Model file for the job. Use its own axes, mm. A direction names the side the tool comes from. Coordinates: 2 decimals unless noted, no trailing zeros. Order: outer loops, then holes, each group sorted by start corner. A loop starts at its lowest first (then second) coordinate and runs counter-clockwise, first axis right, second up.
from build123d import *

# Parameters (mm, degrees)
BASE_PLATE_SKETCH_W = 88
BASE_PLATE_SKETCH_H = 110
BASE_PLATE_DEPTH    = 18
SIDE_BOSS_SKETCH_W  = 88
SIDE_BOSS_SKETCH_H  = 6
SIDE_BOSS_DEPTH     = 75
REAR_BOSS_SKETCH_R  = 9.5
REAR_BOSS_DEPTH     = 12
ANGLED_CUT_REACH    = 137.133
ANGLED_CUT_SKETCH_R = 5
ARCH_CUT_SKETCH_R   = 24
ARCH_CUT_DEPTH      = 93.743251702


with BuildPart() as part:
    # Base Plate Sketch → Base Plate (new body)
    with BuildSketch(Plane.XY):
        with Locations((0, 55)):
            Rectangle(BASE_PLATE_SKETCH_W, BASE_PLATE_SKETCH_H)
    extrude(amount=-BASE_PLATE_DEPTH)

    # Side Boss Sketch → Side Boss (add)
    with BuildSketch(Plane(origin=(0, 0, 0), x_dir=(1, 0, 0), z_dir=(0, 1, 0))):
        with Locations((0, 21)):
            Rectangle(SIDE_BOSS_SKETCH_W, SIDE_BOSS_SKETCH_H)
    extrude(amount=SIDE_BOSS_DEPTH)

    # Rear Boss Sketch → Rear Boss (add)
    with BuildSketch(Plane.XZ):
        with BuildLine():
            Line((-44, -24), (-19.769224603, -55.302867659))
            ThreePointArc((-19.769224603, -55.302867659), (0, -65), (19.769224603, -55.302867659))
            Line((19.769224603, -55.302867659), (44, -24))
            Line((44, -24), (-44, -24))
        make_face()
        with Locations(Location((0, -40, 0), (0, 0, 270))):
            Circle(REAR_BOSS_SKETCH_R, mode=Mode.SUBTRACT)
    extrude(amount=-REAR_BOSS_DEPTH)

    # Angled Cut: up to this face of the body (flat: up to its plane)
    angled_cut_end = Plane(part.part.faces().sort_by_distance((0, 43.5, -24))[0])
    # Angled Cut Sketch → Angled Cut (cut, up to the picked face)
    with BuildSketch(Plane.XY, mode=Mode.PRIVATE) as angled_cut_sk1:
        with Locations((-27.5, 95)):
            Circle(ANGLED_CUT_SKETCH_R)
    angled_cut_tool1 = split(extrude(angled_cut_sk1.sketch, amount=-ANGLED_CUT_REACH, mode=Mode.PRIVATE), bisect_by=angled_cut_end, keep=Keep.BOTH, mode=Mode.PRIVATE)
    # Angled Cut Sketch → Angled Cut (cut, up to the picked face)
    with BuildSketch(Plane.XY, mode=Mode.PRIVATE) as angled_cut_sk2:
        with Locations((27.5, 95)):
            Circle(ANGLED_CUT_SKETCH_R)
    angled_cut_tool2 = split(extrude(angled_cut_sk2.sketch, amount=-ANGLED_CUT_REACH, mode=Mode.PRIVATE), bisect_by=angled_cut_end, keep=Keep.BOTH, mode=Mode.PRIVATE)
    # Angled Cut Sketch → Angled Cut (cut, up to the picked face)
    with BuildSketch(Plane.XY, mode=Mode.PRIVATE) as angled_cut_sk3:
        with Locations((29.652920455, 60)):
            Circle(ANGLED_CUT_SKETCH_R)
    angled_cut_tool3 = split(extrude(angled_cut_sk3.sketch, amount=-ANGLED_CUT_REACH, mode=Mode.PRIVATE), bisect_by=angled_cut_end, keep=Keep.BOTH, mode=Mode.PRIVATE)
    # Angled Cut Sketch → Angled Cut (cut, up to the picked face)
    with BuildSketch(Plane.XY, mode=Mode.PRIVATE) as angled_cut_sk4:
        with Locations((-29.652920455, 60)):
            Circle(ANGLED_CUT_SKETCH_R)
    angled_cut_tool4 = split(extrude(angled_cut_sk4.sketch, amount=-ANGLED_CUT_REACH, mode=Mode.PRIVATE), bisect_by=angled_cut_end, keep=Keep.BOTH, mode=Mode.PRIVATE)
    add(angled_cut_tool1.solids().sort_by(Axis((-27.5, 95, 0), (0, 0, -1)))[0], mode=Mode.SUBTRACT)
    add(angled_cut_tool2.solids().sort_by(Axis((27.5, 95, 0), (0, 0, -1)))[0], mode=Mode.SUBTRACT)
    add(angled_cut_tool3.solids().sort_by(Axis((29.65292, 60, 0), (0, 0, -1)))[0], mode=Mode.SUBTRACT)
    add(angled_cut_tool4.solids().sort_by(Axis((-29.65292, 60, 0), (0, 0, -1)))[0], mode=Mode.SUBTRACT)

    # Arch Cut Sketch → Arch Cut (cut, along a direction that is not the sketch's normal)
    with BuildSketch(Plane.XZ):
        Circle(ARCH_CUT_SKETCH_R)
    extrude(amount=-ARCH_CUT_DEPTH, dir=(0, -0.9063077870366493, -0.4226182617407009), mode=Mode.SUBTRACT)


solid = part.part
Q1. Mould opens along Z. For faces 3 (the face through (-1, 68, 0)), 4 (the face through (-3.639, 5.916, -48.776)), 5 (the face through (32.341, 64.216, -11.832)), 6 (the face through (-1, 43, -24)) say: pulls with the +Z half, pulls with the -Z half, needs draft (parallel to the pull), parting line crosses it, or undercut.
Established:
face 3: pulls with the +Z half
face 4: undercut
face 5: needs draft
face 6: pulls with the -Z half
Q2. Which spindle directions (+Z, -Z, +X, -X, +Y, -Y) get a long thin tool onto all of the face, cutting with end or side? Do faces 1 (the face through (-33.34, 63.38, -11.83)), 2 (the face through (-1, 75, -21)). Say none if no direction does.
Established:
face 1: +Z, -Z
face 2: -Z, +X, -X, +Y
Q3. Cut at B-B, the plane z = -40. List the corners of the cut face in (x, y).
Established:
outline: (-31.61, 0) - (-9.5, 0) - (-9.5, 12) - (-31.61, 12) - close; (9.5, 0) - (31.61, 0) - (31.61, 12) - (9.5, 12) - close
Q4. Cut at D-D, the plane x = 36.5. List the corners of the cut face in (y, z), plus the area to 3 significant figures.
Established:
outline: (0, -33.69) - (12, -33.69) - (12, -24) - (75, -24) - (75, -18) - (110, -18) - (110, 0) - (0, 0) - close
area: 2,550 mm2
Q5. Drop flat-ended pins along their axis: P1, Ø19, axis at x = -15.5, y = 44.5, coming from the -Z side; P2, Ø10, axis at x = -31.5, y = 93.5, coming from the -Z side; P3, Ø20.5, axis at x = -14.5, z = -47.5, coming from the +Y side. Give the stop position or say it passes through.
Established:
P1: stops at z = -24
P2: stops at z = -18
P3: stops at y = 12
Q6. Cut at A-A, the plane y = 60. List the corners of the cut face in (x, z), plus the area to 3 significant figures.
Established:
outline: (-44, -24) - (-34.65, -24) - (-34.65, 0) - (-44, 0) - close; (-24.65, -24) - (24.65, -24) - (24.65, 0) - (-24.65, 0) - close; (34.65, -24) - (44, -24) - (44, 0) - (34.65, 0) - close
area: 1,630 mm2
Q7. Cut at C-C, the plane x = -27.5. List the corners of the cut face in (y, z), plus the area to 3 significant figures.
Established:
outline: (0, -45.32) - (12, -45.32) - (12, -24) - (55.49, -24) - (55.49, 0) - (0, 0) - close; (64.51, -24) - (75, -24) - (75, -18) - (90, -18) - (90, 0) - (64.51, 0) - close; (100, -18) - (110, -18) - (110, 0) - (100, 0) - close
area: 2,290 mm2
Q8. Probe line 1 (Y direction, x = -27, z = -3); line 2 (X direction, y = 64, z = -16.5); line 3 (Y direction, x = -27.5, z = -4.75). List the from-to ranges inside material, lowest first.
Established:
line 1: y = 0 to 55.76, 64.24 to 90.03, 99.97 to 110
line 2: x = -44 to -32.65, -26.65 to 26.65, 32.65 to 44
line 3: y = 0 to 55.49, 64.51 to 90, 100 to 110
